```python
from build123d import *

# Parameters (mm, degrees)
EXTRUDE1_DEPTH            = 65
SKETCH2_R                 = 16
EXTRUDE2_DEPTH            = 6
EXTRUDE3_START            = -6
SKETCH3_R                 = 16
EXTRUDE3_DEPTH            = 6
M5X0_8_TAPPED_HOLE1_D     = 4.2
M5X0_8_TAPPED_HOLE1_DEPTH = 12.4
M5X0_8_TAPPED_HOLE1_TIP   = 1.2618073
M4X0_7_TAPPED_HOLE1_D     = 3.3
M4X0_7_TAPPED_HOLE1_DEPTH = 10.1
M4X0_7_TAPPED_HOLE1_TIP   = 0.991420021


with BuildPart() as part:
    # Sketch1 → Extrude1 (new body)
    with BuildSketch(Plane(origin=(0, 0, 0), x_dir=(0, 0, -1), z_dir=(1, 0, 0))):
        with BuildLine():
            Line((-23.5, -25), (-9.449924117, -25))
            Line((-9.449924117, -25), (-4, -11.842719282))
            ThreePointArc((-4, -11.842719282), (0, 12.5), (4, -11.842719282))
            Line((4, -11.842719282), (9.449924117, -25))
            Line((9.449924117, -25), (23.5, -25))
            Line((23.5, -25), (23.5, 8))
            Line((23.5, 8), (25, 8))
            Line((25, 8), (25, 22))
            Line((25, 22), (8, 22))
            Line((8, 22), (8, 21))
            Line((8, 21), (-8, 21))
            Line((-8, 21), (-8, 22))
            Line((-8, 22), (-25, 22))
            Line((-25, 22), (-25, 8))
            Line((-25, 8), (-23.5, 8))
            Line((-23.5, 8), (-23.5, -25))
        make_face()
    extrude(amount=EXTRUDE1_DEPTH)

    # Sketch2 → Extrude2 (cut)
    with BuildSketch(Plane(origin=(65, 0, 0), x_dir=(0, 0, -1), z_dir=(1, 0, 0))):
        Circle(SKETCH2_R)
    extrude(amount=-EXTRUDE2_DEPTH, mode=Mode.SUBTRACT)

    # Sketch3 → Extrude3 (cut)
    with BuildSketch(Plane.ZY.offset(EXTRUDE3_START)):
        Circle(SKETCH3_R)
    extrude(amount=EXTRUDE3_DEPTH, mode=Mode.SUBTRACT)

    # M5x0.8 Tapped Hole1
    with Locations(Plane(origin=(12.5, 22, -20), x_dir=(0, 0, 1), z_dir=(0, 1, 0))):
        with Locations((0, 0), (0, 40), (40, 0), (40, 40)):
            Hole(M5X0_8_TAPPED_HOLE1_D / 2, depth=M5X0_8_TAPPED_HOLE1_DEPTH)
            with Locations((0, 0, -(M5X0_8_TAPPED_HOLE1_DEPTH + M5X0_8_TAPPED_HOLE1_TIP / 2))):  # 118° drill point
                Cone(0, M5X0_8_TAPPED_HOLE1_D / 2, M5X0_8_TAPPED_HOLE1_TIP, mode=Mode.SUBTRACT)

    # M4x0.7 Tapped Hole1
    with Locations(Plane(origin=(32.5, 22, 0), x_dir=(0, 0, 1), z_dir=(0, 1, 0))):
        with Locations((0, 0)):
            Hole(M4X0_7_TAPPED_HOLE1_D / 2, depth=M4X0_7_TAPPED_HOLE1_DEPTH)
            with Locations((0, 0, -(M4X0_7_TAPPED_HOLE1_DEPTH + M4X0_7_TAPPED_HOLE1_TIP / 2))):  # 118° drill point
                Cone(0, M4X0_7_TAPPED_HOLE1_D / 2, M4X0_7_TAPPED_HOLE1_TIP, mode=Mode.SUBTRACT)


solid = part.part
```
Here's how the part is built. I have some questions about the finished solid (model axes, mm). A direction names the side the tool comes from. Give positions to 0.01 mm unless a question says otherwise; leave off trailing zeros. Loops run counter-clockwise (first coordinate to the right, second up) from the corner with the lowest first, then second, coordinate; pieces in that order, holes last. Notation, with made-up numbers: M 55,76.25 L 114,76.25 A17 ccw 114,109.25 Z; hole C -20,-0.75 d2. An arc over 180 degrees is marked long. Put each result on its own line as item: value. Start each with the question number.
(1) I want a section at D-D on x = 24.5. Please give me the cut outline in (y, z), then the cut area to 3 significant figures.
(2) I want a section at A-A on x = 32.5. Please give me the cut outline in (y, z), then the cut area to 3 significant figures.
(3) I want a section at C-C on y = -19. Please give me the cut outline in (x, z).
(4) If we mould it in two halves opening along X, with no side actions, what happens to faces 1 (the flat face through (65, -12, 11)), 2 (the cylindrical face through (50.637, 15.713, 19.031)), 3 (the flat face through (32, 15, -25))? For each: +X half, -X half, draft (parallel to the pull), parting line (faces both ways), or undercut.
(5) For faces 4 (the cylindrical face through (62.042, 15.988, -0.627)), 5 (the cylindrical face through (13.131, 15.713, -22.003)), 6 (the flat face through (32.045, -18.329, -6.687)), 7 (the flat face through (32, -8, 23.5)), 8 (the flat face through (32, -9, -23.5)), which set-ups out of +Z, -Z, +X, -X, +Y, -Y let a thin tool reach every point of the face, with its end or its side?
(6) I need wall thicknesses on line 1 along X through (y, z) = (18.75, 20); line 2 along Z through (x, y) = (12, 19); line 3 along Z through (x, y) = (42, 0). Which ranges of each line are inside material? Lowest first, please. Write a range as [from, to].
(7) Will these pins go through, and if not, where does the flat tip stop? pin 1 Ø5.5 at (x, z) = (32.5, 0) entering from -Y; pin 2 Ø1.5 at (x, y) = (17.5, -10) entering from +Z; pin 3 Ø5 at (x, z) = (24.5, -3.5) entering from +Y.
(8) I want a section at B-B on y = 19. Please give me the cut outline in (x, z).
Answer block:
1. outline: M -25,-23.5 L 8,-23.5 L 8,-25 L 22,-25 L 22,-8 L 21,-8 L 21,8 L 22,8 L 22,25 L 8,25 L 8,23.5 L -25,23.5 L -25,9.45 L -11.84,4 A12.5 cw long -11.84,-4 L -25,-9.45 Z
1. area: 1,570 mm^2
2. outline: M -25,-23.5 L 8,-23.5 L 8,-25 L 22,-25 L 22,-8 L 21,-8 L 21,-1.65 L 12.39,-1.65 A12.5 cw -11.84,-4 L -25,-9.45 Z; M -25,9.45 L -11.84,4 A12.5 cw 12.39,1.65 L 21,1.65 L 21,8 L 22,8 L 22,25 L 8,25 L 8,23.5 L -25,23.5 Z
2. area: 1,540 mm^2
3. outline: M 0,-23.5 L 65,-23.5 L 65,-6.96 L 0,-6.96 Z; M 0,6.96 L 65,6.96 L 65,23.5 L 0,23.5 Z
4. face 1: +X half
4. face 2: undercut
4. face 3: draft
5. face 4: +X
5. face 5: +Y
5. face 6: +X, -X, -Y
5. face 7: +Z, +X, -X, -Y
5. face 8: -Z, +X, -X, -Y
6. line 1: [0, 10.4], [14.6, 50.4], [54.6, 65]
6. line 2: [-25, -22.04], [-17.96, 17.96], [22.04, 25]
6. line 3: [-23.5, -12.5], [12.5, 23.5]
7. pin 1: y = 12.19
7. pin 2: z = 23.5
7. pin 3: y = 21
8. outline: M 0,-25 L 65,-25 L 65,25 L 0,25 Z; hole C 12.5,-20 d4.2; hole C 12.5,20 d4.2; hole C 32.5,0 d3.3; hole C 52.5,-20 d4.2; hole C 52.5,20 d4.2
